Geometry: final body of the model. Coordinates: model frame, mm. A direction names the side the tool comes from. Coordinates: 2 decimals unless noted, no trailing zeros. Write each loop counter-clockwise with the first axis right and the second up, starting at its lowest first coordinate (ties: lowest second). Pieces come first, ordered by that corner, then holes. Notation, with made-up numbers: (-37, -38) - (2, -38) arc R8 ccw to (2, -24) - close; hole circle Ø6 at (-2, 28.5). An arc over 180 degrees is marked (long way). Put each result on its own line as item: value.
```python
from build123d import *

# Parameters (mm, degrees)
SKETCH_1_R             = 2.5
EXTRUDE_1_DEPTH        = 15
HOLE_WIZARD_M3_1_D     = 2.5
HOLE_WIZARD_M3_1_DEPTH = 7.5
HOLE_WIZARD_M3_1_TIP   = 0.751075774
CHAMFER_1_SIZE         = 0.5


with BuildPart() as part:
    # 草图1 → 凸台-拉伸1 (new body)
    with BuildSketch(Plane(origin=(0, 0, 0), x_dir=(1, 0, 0), z_dir=(0, 1, 0))):
        with Locations(Location((0, 0, 0), (0, 0, 270))):
            Circle(SKETCH_1_R)
    extrude(amount=EXTRUDE_1_DEPTH)

    # M3 螺纹孔1
    with Locations(Plane(origin=(0, 0, 0), x_dir=(-1, 0, 0), z_dir=(0, -1, 0))):
        with Locations((0, 0)):
            Hole(HOLE_WIZARD_M3_1_D / 2, depth=HOLE_WIZARD_M3_1_DEPTH)
            with Locations((0, 0, -(HOLE_WIZARD_M3_1_DEPTH + HOLE_WIZARD_M3_1_TIP / 2))):  # 118° drill point
                Cone(0, HOLE_WIZARD_M3_1_D / 2, HOLE_WIZARD_M3_1_TIP, mode=Mode.SUBTRACT)

    # 倒角1
    chamfer_1_edges = [part.edges().sort_by_distance(p)[0] for p in [
        (0, 0, -2.5),
        (0, 15, -2.5),
    ]]
    chamfer(chamfer_1_edges, length=CHAMFER_1_SIZE)


solid = part.part
```
1. Pin query (flat end, axial travel): pin 1 Ø1.5 at (x, y) = (-1.5, 6.5) entering from -Z. Return the tip coordinate at first contact, or that it passes through.
Answer below:
pin 1: stops at z = -2.38
2. Mould query, pull axis Z, two halves, no side actions, for faces 1 (the flat face through (1, 0, 1)), 2 (the cylindrical face through (-2.44, 7.4, -0.54)), 3 (the conical face through (0.05, 8.12, 0.21)). Classes: +Z half, -Z half, draft (parallel to the pull), parting line (faces both ways), or undercut.
Answer below:
face 1: draft
face 2: parting line
face 3: undercut
3. Section query B-B (y = 12.5). Return loops of the section in (x, z).
Answer below:
outline: circle Ø5 at (0, 0)
4. Ray query, probe 1 along Z at (x, y) = (0.1, 6.25); probe 2 along X at (y, z) = (3.75, -0.75); probe 3 along Z at (x, y) = (-1, 5). Return the intervals inside material, ascending. Write a range as from..to.
Answer below:
probe 1: z = -2.5..-1.25, 1.25..2.5
probe 2: x = -2.38..-1, 1..2.38
probe 3: z = -2.29..-0.75, 0.75..2.29
5. Section query A-A (y = 3.25). Return loops of the section in (x, z), then the cut area to 3 significant figures.
Answer below:
outline: circle Ø5 at (0, 0); hole circle Ø2.5 at (0, 0)
area: 14.7 mm²
6. Set-up query: faces 4 (the cylindrical face through (-0.27, 3.8, 1.22)), 5 (the flat face through (0, 15, 0)). Return all of +Z, -Z, +X, -X, +Y, -Y with unobstructed straight access to the full face (end or side cutting, diameter ignored); none if empty.
Answer below:
face 4: -Y
face 5: +Z, -Z, +X, -X, +Y
